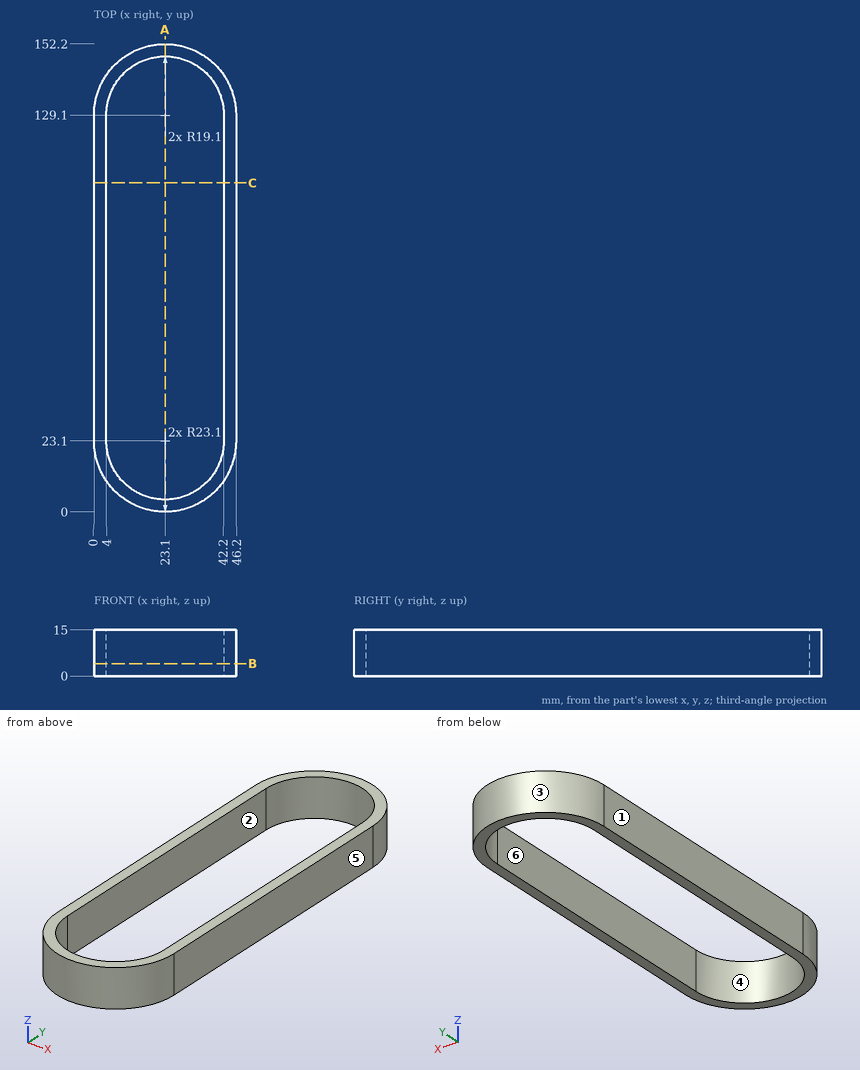
Job drawing, mm, ordinate dimensions from the low corner. One solid piece. A direction names the side the tool comes from. Give positions to 0.01 mm unless a question says otherwise; leave off trailing zeros. Loops run counter-clockwise (first coordinate to the right, second up) from the corner with the lowest first, then second, coordinate; pieces in that order, holes last. Notation, with made-up numbers: M -22,-31 L 9,-31 A28 cw 9,-9 Z; hole C 38.25,38 d6. An arc over 180 degrees is marked long. Put each result on its own line as item: value. Start each with the question number.
1) Flat gauge pins, fed straight in: pin 1 (4 mm diameter, centred on y = 133.5, z = 9.5, fed in from -X) (3 decimals); pin 2 (1 mm diameter, centred on y = 129.5, z = 8, fed in from +X); pin 3 (2 mm diameter, centred on x = 17, z = 10, fed in from -Y); pin 4 (2 mm diameter, centred on x = 33, z = 9.5, fed in from -Y). Where does each tip first touch, or does it go through?
2) Saw through at C-C (y = 107). List the corners of the cut face in (x, z).
3) Pull direction X, two halves, no side cores. Call the marked faces 1, 2, 3 and 4: +X half, -X half, draft (parallel to the pull), parting line (faces both ways), or undercut.
4) Saw through at B-B (z = 4). List the corners of the cut face in (x, y), then the cut area to 3 significant figures.
5) Saw through at A-A (x = 23.1). List the corners of the cut face in (y, z), then the cut area to 3 significant figures.
6) Probe probe 1 along X at (y, z) = (113.5, 14); probe 2 along Y at (x, z) = (12.5, 10); probe 3 along Y at (x, z) = (24.5, 4.25). List the from-to ranges inside material, lowest first.
7) 3-axis set-ups, long thin cutter, end or side, ignore diameter. For the marked faces 5 and 6: which of +Z, -Z, +X, -X, +Y, -Y reach the whole face in a straight line?
Numbers:
1. pin 1: x = 0.125
1. pin 2: x = 46.2
1. pin 3: y = 0.57
1. pin 4: y = 1.78
2. outline: M 0,0 L 4,0 L 4,15 L 0,15 Z; M 42.2,0 L 46.2,0 L 46.2,15 L 42.2,15 Z
3. face 1: -X half
3. face 2: undercut
3. face 3: parting line
3. face 4: undercut
4. outline: M 0,23.1 A23.1 ccw 46.2,23.1 L 46.2,129.1 A23.1 ccw 0,129.1 Z; hole M 4,23.1 A19.1 ccw 42.2,23.1 L 42.2,129.1 A19.1 ccw 4,129.1 Z
4. area: 1,380 mm^2
5. outline: M 0,0 L 4,0 L 4,15 L 0,15 Z; M 148.2,0 L 152.2,0 L 152.2,15 L 148.2,15 Z
5. area: 120 mm^2
6. probe 1: 0 to 4, 42.2 to 46.2
6. probe 2: 2.58 to 7.21, 144.99 to 149.62
6. probe 3: 0.04 to 4.05, 148.15 to 152.16
7. face 5: +Z, -Z, +X, +Y, -Y
7. face 6: +Z, -Z
